from build123d import *

# Parameters (mm, degrees)
EXTRUDE_1_DEPTH = 30


with BuildPart() as part:
    # 草图1 → 凸台-拉伸1 (new body)
    with BuildSketch(Plane(origin=(0, 0, 0), x_dir=(1, 0, 0), z_dir=(0, 1, 0))):
        Polygon((0, 0), (-30, 0), (-220, -109.696551146), (-220, -139.696551146), (-20, -139.696551146), (0, -119.696551146), align=None)
    extrude(amount=EXTRUDE_1_DEPTH)


solid = part.part
Design review of the part built by this model. Coordinates are the model's own, in mm. Coordinates: 2 decimals unless noted, no trailing zeros. Write each loop counter-clockwise with the first axis right and the second up, starting at its lowest first coordinate (ties: lowest second). Pieces come first, ordered by that corner, then holes. Notation, with made-up numbers: (50, -34) - (95, -34) arc R11 cw to (95, -22) - close; hole circle Ø4 at (-12, 24.25). An arc over 180 degrees is marked (long way). Use one line per item in the form item = value.
Q1. For probe 1 along X at (y, z) = (10.5, 56.5); probe 2 along X at (y, z) = (24, 36.5); probe 3 along Z at (x, y) = (-166, 19.5), list the stretches that pass through material, from the lowest coordinate up.
Taken from the geometry:
probe_1 = -127.86 to 0
probe_2 = -93.22 to 0
probe_3 = 78.52 to 139.7
Q2. Insertion check: pin 1 Ø3 at (y, z) = (11.5, 75) entering from +X; pin 2 Ø3 at (x, y) = (-187, 7.5) entering from -Z; pin 3 Ø8 at (y, z) = (12, 85) entering from -X. Each pin has a flat end and moves straight along its axis. Give the tip position at first contact, or say it passes through.
Taken from the geometry:
pin_1 = 0
pin_2 = 89.78
pin_3 = -184.15
Q3. The part is to be moulded in two halves that separate along X. For faces 1 (the flat face through (0, 15, 61)), 2 (the flat face through (-123.7, 14.8, 54.1)), 3 (the flat face through (-15, 15, 0)), say which applies: +X half, -X half, draft (parallel to the pull), parting line (faces both ways), or undercut.
Taken from the geometry:
face_1 = +X half
face_2 = -X half
face_3 = draft
Q4. Consider section C-C (x = -158). Write out the cut boundary in (y, z).
Taken from the geometry:
outline = (0, 73.9) - (30, 73.9) - (30, 139.7) - (0, 139.7) - close
Q5. Consider section B-B (z = 69). Write out the cut boundary in (x, y).
Taken from the geometry:
outline = (-149.51, 0) - (0, 0) - (0, 30) - (-149.51, 30) - close
Q6. Consider section A-A (y = 6.5). Write out the cut boundary in (x, z).
Taken from the geometry:
outline = (-220, 109.7) - (-30, 0) - (0, 0) - (0, 119.7) - (-20, 139.7) - (-220, 139.7) - close
